```python
from build123d import *

# Parameters (mm, degrees)
SKETCH_1_W               = 34
SKETCH_1_H               = 19.5
EXTRUDE_1_DEPTH          = 28.4
CUT_EXTRUDE_1_DEPTH      = 35.505398128
CUT_EXTRUDE_1_DEPTH_BACK = 35.505398128
SKETCH_2_W               = 15
SKETCH_2_H               = 10.5
SKETCH_4_R               = 1.8
CUT_EXTRUDE_2_DEPTH      = 6


with BuildPart() as part:
    # 草图1 → 凸台-拉伸1 (new, symmetric)
    with BuildSketch(Plane.XY):
        Rectangle(SKETCH_1_W, SKETCH_1_H)
    extrude(amount=EXTRUDE_1_DEPTH, both=True)

    # 草图2 → 切除-拉伸1 (cut, two sides: drawn at the far end of the back side and taken through both)
    with BuildSketch(Plane.XY.offset(-CUT_EXTRUDE_1_DEPTH_BACK)):
        with Locations((0, -4.5)):
            Rectangle(SKETCH_2_W, SKETCH_2_H)
    extrude(amount=CUT_EXTRUDE_1_DEPTH + CUT_EXTRUDE_1_DEPTH_BACK, mode=Mode.SUBTRACT)

    # 草图4 → 切除-拉伸2 (cut)
    with BuildSketch(Plane(origin=(0, 9.75, 0), x_dir=(1, 0, 0), z_dir=(0, 1, 0))):
        with Locations(Location((-13, 13, 0), (0, 0, 270))):
            Circle(SKETCH_4_R)
        with Locations(Location((13, 13, 0), (0, 0, 90))):
            Circle(SKETCH_4_R)
        with Locations(Location((13, -13, 0), (0, 0, 270))):
            Circle(SKETCH_4_R)
        with Locations(Location((-13, -13, 0), (0, 0, 90))):
            Circle(SKETCH_4_R)
    extrude(amount=-CUT_EXTRUDE_2_DEPTH, mode=Mode.SUBTRACT)


solid = part.part
```
For this review, take the finished solid that the model builds, in its own axes (mm). A direction names the side the tool comes from. Give positions to 0.01 mm unless a question says otherwise; leave off trailing zeros. Order: outer loops, then holes, each group sorted by start corner. A loop starts at its lowest first (then second) coordinate and runs counter-clockwise, first axis right, second up.
1) Wall thickness on line 1 (X direction, y = 6.9, z = -13); line 2 (X direction, y = -6.75, z = -23); line 3 (Y direction, x = -6, z = -14): over which ranges is each line inside the solid? List them lowest first.
2) For faces 1 (the face through (0, 0.75, 0)), 2 (the face through (14.217, 6.792, 11.673)), 3 (the face through (0, 2, 28.4)), list the 3-axis set-ups (+Z, -Z, +X, -X, +Y, -Y) from which the entire face can be reached by the end or side of a thin tool; tool diameter is ignored.
3) Take a section at C-C (y = 5.5). Give the boundary of the cut face in (x, z), then the cut area to 3 significant figures.
4) The part is to be moulded in two halves that separate along X. For faces 4 (the face through (7.5, -5, 0)), 5 (the face through (-13, 3.75, 13)), 6 (the face through (12, -9.75, 0)), 7 (the face through (-17, 0, 0)), say which applies: released by +X, released by -X, zero draft, split by the parting line, or undercut.
5) Take a section at D-D (x = -13). Give the boundary of the cut face in (y, z).
6) Insertion check: pin 1 (5 mm diameter, centred on x = -3, z = 16.5, fed in from -Y); pin 2 (1.1 mm diameter, centred on x = 12, z = -13.5, fed in from +Y); pin 3 (3 mm diameter, centred on x = 13.5, z = 13, fed in from +Y). Each pin has a flat end and moves straight along its axis. Give the tip position at first contact, or say it passes through.
7) Take a section at A-A (y = -3.5). Give the boundary of the cut face in (x, z), then the cut area to 3 significant figures.
8) Take a section at B-B (z = 16). Give the boundary of the cut face in (x, y).
Derived:
1. line 1: x = -17 to -14.8, -11.2 to 11.2, 14.8 to 17
1. line 2: x = -17 to -7.5, 7.5 to 17
1. line 3: y = 0.75 to 9.75
2. face 1: +Z, -Z, -Y
2. face 2: +Y
2. face 3: +Z, +X, -X, +Y, -Y
3. outline: (-17, -28.4) - (17, -28.4) - (17, 28.4) - (-17, 28.4) - close; hole circle Ø3.6 at (-13, -13); hole circle Ø3.6 at (-13, 13); hole circle Ø3.6 at (13, -13); hole circle Ø3.6 at (13, 13)
3. area: 1,890 mm2
4. face 4: undercut
4. face 5: undercut
4. face 6: zero draft
4. face 7: released by -X
5. outline: (-9.75, -28.4) - (9.75, -28.4) - (9.75, -14.8) - (3.75, -14.8) - (3.75, -11.2) - (9.75, -11.2) - (9.75, 11.2) - (3.75, 11.2) - (3.75, 14.8) - (9.75, 14.8) - (9.75, 28.4) - (-9.75, 28.4) - close
6. pin 1: stops at y = 0.75
6. pin 2: stops at y = 3.75
6. pin 3: stops at y = 9.75
7. outline: (-17, -28.4) - (-7.5, -28.4) - (-7.5, 28.4) - (-17, 28.4) - close; (7.5, -28.4) - (17, -28.4) - (17, 28.4) - (7.5, 28.4) - close
7. area: 1,080 mm2
8. outline: (-17, -9.75) - (-7.5, -9.75) - (-7.5, 0.75) - (7.5, 0.75) - (7.5, -9.75) - (17, -9.75) - (17, 9.75) - (-17, 9.75) - close
